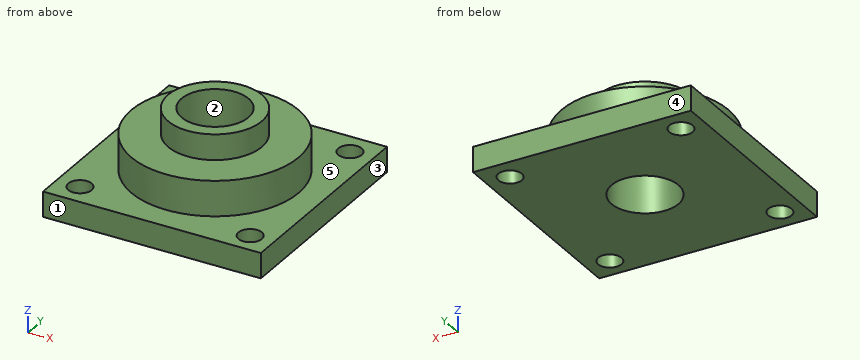
from build123d import *

# Parameters (mm, degrees)
FLANGE_PLATE_SKETCH_W         = 130
FLANGE_PLATE_SKETCH_H         = 130
FLANGE_PLATE_130X130X15_DEPTH = 15
HUB_SKETCH_100_R              = 50
HUB_100_DEPTH                 = 21
SPIGOT_SKETCH_56_R            = 28
SPIGOT_56_DEPTH               = 15.2
BORE_SKETCH_40_R              = 20
BORE_40_DEPTH                 = 51.2
MOUNTING_HOLES_SKETCH_R       = 7
MOUNTING_HOLES_4X_14_DEPTH    = 15


with BuildPart() as part:
    # Flange Plate Sketch → Flange Plate 130x130x15 (new body)
    with BuildSketch(Plane.XY):
        with Locations((65, 65)):
            Rectangle(FLANGE_PLATE_SKETCH_W, FLANGE_PLATE_SKETCH_H)
    extrude(amount=FLANGE_PLATE_130X130X15_DEPTH)

    # Hub Sketch Ø100 → Hub Ø100 (add)
    with BuildSketch(Plane.XY.offset(15)):
        with Locations(Location((65, 65, 0), (0, 0, 180))):
            Circle(HUB_SKETCH_100_R)
    extrude(amount=HUB_100_DEPTH)

    # Spigot Sketch Ø56 → Spigot Ø56 (add)
    with BuildSketch(Plane.XY.offset(36)):
        with Locations(Location((65, 65, 0), (0, 0, 180))):
            Circle(SPIGOT_SKETCH_56_R)
    extrude(amount=SPIGOT_56_DEPTH)

    # Bore Sketch Ø40 → Bore Ø40 (cut)
    with BuildSketch(Plane.XY.offset(51.2)):
        with Locations((65, 65)):
            Circle(BORE_SKETCH_40_R)
    extrude(amount=-BORE_40_DEPTH, mode=Mode.SUBTRACT)

    # Mounting Holes Sketch → Mounting Holes 4xØ14 (cut)
    with BuildSketch(Plane.XY.offset(15)):
        with Locations((116, 116)):
            Circle(MOUNTING_HOLES_SKETCH_R)
        with Locations((14, 116)):
            Circle(MOUNTING_HOLES_SKETCH_R)
        with Locations((14, 14)):
            Circle(MOUNTING_HOLES_SKETCH_R)
        with Locations((116, 13.196511798)):
            Circle(MOUNTING_HOLES_SKETCH_R)
    extrude(amount=-MOUNTING_HOLES_4X_14_DEPTH, mode=Mode.SUBTRACT)


solid = part.part
Part model, mm, in its own coordinate system. Face numbers are marked on the shaded views. A direction names the side the tool comes from. Coordinates: 2 decimals unless noted, no trailing zeros. Loops run counter-clockwise (first coordinate to the right, second up) from the corner with the lowest first, then second, coordinate; pieces in that order, holes last. Notation, with made-up numbers: M -34.5,88.5 L 13.5,88.5 A22 cw 13.5,127.5 Z; hole C -20.5,51.25 d9. An arc over 180 degrees is marked long. Use a Markdown table: item, result. Add a question column.
Q1. Cut at D-D (y = 102.5). Write the cut outline in (x, z).
Q2. Pin check, flat tips, straight feed: P1, Ø8.5, axis at x = 14, y = 14, coming from the +Z side; P2, Ø2, axis at x = 81.5, y = 100.5, coming from the +Z side; P3, Ø10, axis at y = 105, z = 32, coming from the +X side; P4, Ø12, axis at y = 28.5, z = 27, coming from the +X side. Stop position of each tip, or through.
Q3. Cut at A-A (y = 65). Write the cut outline in (x, z).
Q4. Which spindle directions (+Z, -Z, +X, -X, +Y, -Y) get a long thin tool onto all of the face, cutting with end or side? Do the marked faces 4 and 5. Say none if no direction does.
Q5. Mould opens along Y. For the marked faces 1, 2 and 3 say: +Y half, -Y half, draft (parallel to the pull), parting line (faces both ways), or undercut.
Q6. Probe L1, parallel to Y at x = 116, z = 7.25; L2, parallel to Y at x = 14, z = 3.5; L3, parallel to Z at x = 27, y = 90. List the from-to ranges inside material, lowest first.
Q7. Cut at C-C (z = 6). Write the cut outline in (x, y).
Worked out:
| question | item | result |
|---|---|---|
| 1 | outline | M 0,0 L 130,0 L 130,15 L 98.07,15 L 98.07,36 L 31.93,36 L 31.93,15 L 0,15 Z |
| 2 | P1 | passes through |
| 2 | P2 | stops at z = 36 |
| 2 | P3 | stops at x = 100.71 |
| 2 | P4 | stops at x = 104.62 |
| 3 | outline | M 0,0 L 45,0 L 45,51.2 L 37,51.2 L 37,36 L 15,36 L 15,15 L 0,15 Z; M 85,0 L 130,0 L 130,15 L 115,15 L 115,36 L 93,36 L 93,51.2 L 85,51.2 Z |
| 4 | face 4 | +Z, -Z, +X, -X, +Y |
| 4 | face 5 | +Z |
| 5 | face 1 | -Y half |
| 5 | face 2 | undercut |
| 5 | face 3 | draft |
| 6 | L1 | y = 0 to 6.2, 20.2 to 109, 123 to 130 |
| 6 | L2 | y = 0 to 7, 21 to 109, 123 to 130 |
| 6 | L3 | z = 0 to 36 |
| 7 | outline | M 0,0 L 130,0 L 130,130 L 0,130 Z; hole C 14,14 d14; hole C 14,116 d14; hole C 65,65 d40; hole C 116,13.2 d14; hole C 116,116 d14 |
